from build123d import *

# Parameters (mm, degrees)
BOLT_HOLES_SKETCH_R        = 6.25
FLANGE_BOLT_HOLES_4X_DEPTH = 52
FILLET_R3_5_R              = 3.5
FILLET_R1_R                = 1


with BuildPart() as part:
    # Connector Profile Sketch → Connector Body Revolve (revolve)
    with BuildSketch(Plane.XY, mode=Mode.PRIVATE) as connector_body_revolve_sk:
        Polygon((0, 25), (30, 25), (30, 20), (74.2, 20), (74.2, 75.14842088), (88.4, 75.14842088), (88.4, 15), (24, 15), (24, 20), (0, 20), align=None)
    revolve(connector_body_revolve_sk.sketch.rotate(Axis((-1000, 0, 0), (1, 0, 0)), 90), axis=Axis((-1000, 0, 0), (1, 0, 0)))

    # Bolt Holes Sketch → Flange Bolt Holes 4x (cut)
    with BuildSketch(Plane.ZY.offset(-74.2)):
        with Locations((0, 60.5)):
            Circle(BOLT_HOLES_SKETCH_R)
        with Locations((0, -60.5)):
            Circle(BOLT_HOLES_SKETCH_R)
        with Locations((-60.5, 0)):
            Circle(BOLT_HOLES_SKETCH_R)
        with Locations((60.5, 0)):
            Circle(BOLT_HOLES_SKETCH_R)
    extrude(amount=-FLANGE_BOLT_HOLES_4X_DEPTH, mode=Mode.SUBTRACT)

    # Fillet R3.5
    fillet_r3_5_edges = [part.edges().sort_by_distance(p)[0] for p in [
        (88.4, 0, -15),
    ]]
    fillet(fillet_r3_5_edges, radius=FILLET_R3_5_R)

    # Fillet R1
    fillet_r1_edges = [part.edges().sort_by_distance(p)[0] for p in [
        (74.2, 0, -75.14842088),
        (74.2, 0, -20),
        (0, 0, -25),
        (88.4, 0, -75.14842088),
    ]]
    fillet(fillet_r1_edges, radius=FILLET_R1_R)


solid = part.part
Design review of the part built by this model. Coordinates are the model's own, in mm. A direction names the side the tool comes from. Give positions to 0.01 mm unless a question says otherwise; leave off trailing zeros. Order: outer loops, then holes, each group sorted by start corner. A loop starts at its lowest first (then second) coordinate and runs counter-clockwise, first axis right, second up.
1. Tool access review of faces 4 (the flat face through (88.4, 15, 15)), 5 (the cylindrical face through (51.9, -0.88, -19.98)), 6 (the cylindrical face through (11.83, -0.88, -19.98)): name each direction out of +Z, -Z, +X, -X, +Y, -Y from which nothing blocks a thin tool from reaching the whole face with its end or side.
Solution:
face 4: +Z, -Z, +X, +Y, -Y
face 5: none
face 6: -X
2. Mouldability with a two-part tool opening along Y and no side actions: class faces 1 (the cylindrical face through (81.2, 1.88, -54.54)), 2 (the cylindrical face through (81.39, -22.57, 71.68)), 3 (the flat face through (0, -20, 5)) as +Y half, -Y half, draft (parallel to the pull), parting line (faces both ways), or undercut.
Solution:
face 1: undercut
face 2: parting line
face 3: draft
3. To check wall thickness, follow L1, parallel to Y at x = 78.75, z = 0; L2, parallel to Y at x = 17.25, z = 0; L3, parallel to X at y = -27, z = 65.5. State the ranges of each line that lie inside material, in increasing order.
Solution:
L1: y = -75.15 to -66.75, -54.25 to -15, 15 to 54.25, 66.75 to 75.15
L2: y = -25 to -20, 20 to 25
L3: x = 74.2 to 88.4
4. Add section B-B, the plane y = 0. State how many separate pieces and enclosed holes the cut face has, then the cut area to 3 significant figures.
Solution:
separate pieces: 4
enclosed holes: 0
area: 2,150 mm2
5. For pin 1 Ø11 at (y, z) = (-60.5, 0) entering from +X; pin 2 Ø8 at (y, z) = (34, 30.5) entering from -X; pin 3 Ø2 at (x, y) = (45.5, -10.5) entering from -Z, all flat-tipped, find the tip position at first contact; note any pin that passes through.
Solution:
pin 1: passes through
pin 2: stops at x = 74.2
pin 3: stops at z = -17.6
6. Add section A-A, the plane x = 79. State the section outline as (y, z) points, then the cut area to 3 significant figures.
Solution:
outline: circle Ø150.3 at (0, 0); hole circle Ø12.5 at (-60.5, 0); hole circle Ø30 at (0, 0); hole circle Ø12.5 at (0, -60.5); hole circle Ø12.5 at (0, 60.5); hole circle Ø12.5 at (60.5, 0)
area: 16,500 mm2
7. Add section D-D, the plane x = 21.5. State the section outline as (y, z) points.
Solution:
outline: circle Ø50 at (0, 0); hole circle Ø40 at (0, 0)
